Read the model definition and answer for the solid it produces. Units are mm, in the model's axes. A direction names the side the tool comes from. Give positions to 0.01 mm unless a question says otherwise; leave off trailing zeros. Write each loop counter-clockwise with the first axis right and the second up, starting at its lowest first coordinate (ties: lowest second). Pieces come first, ordered by that corner, then holes. Notation, with made-up numbers: M 9,12 L 47,12 A6 ccw 47,20 Z; hole C 75,-2.75 d8. An arc over 180 degrees is marked long. Use a Markdown table: item, result. Add a question column.
Item 1: A cutting plane is placed at C-C on x = 159. Determine the outline of the cut face in (y, z), then the cut area to 3 significant figures.
Item 2: The mould has two halves that part along X. Classify faces 6 (the flat face through (85, 104, 25)), 7 (the cylindrical face through (111.23, 152.4, 19.15)), 8 (the cylindrical face through (20, 13, 75)), 9 (the conical face through (78.414, 33.759, 98.87)): pulls with the +X half, pulls with the -X half, needs draft (parallel to the pull), parting line crosses it, or undercut.
Item 3: For faces 1 (the flat face through (35, 15, 74)), 2 (the flat face through (203, 13, 80)), 3 (the flat face through (25, 37, 74)), 4 (the cylindrical face through (32.69, 42.4, 68.46)), 5 (the flat face through (185, 38, 74)), determine the directions among +Z, -Z, +X, -X, +Y, -Y from which every point of the face is accessible in a straight line to the end or side of a thin tool.
Item 4: Consider probe 1 along Z at (x, y) = (35, 47); probe 2 along Z at (x, y) = (177, 46); probe 3 along X at (y, z) = (43, 99). Determine where each line is inside the solid, lowest interval first. Write a range as [from, to].
Item 5: Given P1, Ø10, axis at x = 121, z = 33, coming from the +Y side; P2, Ø4.5, axis at x = 94, z = 69, coming from the +Y side; P3, Ø8, axis at x = 78, z = 99, coming from the -Y side; P4, Ø7.5, axis at x = 6, y = 15.5, coming from the -Z side, each flat-ended and moving along its own axis, determine where each tip first touches the part or whether it passes through.
Item 6: A cutting plane is placed at A-A on z = 40. Determine the outline of the cut face in (x, y).
Item 7: A cutting plane is placed at B-B on z = 120. Determine the outline of the cut face in (x, y), then the cut area to 3 significant figures.
from build123d import *

# Parameters (mm, degrees)
BOSS_EXTRUDE1_DEPTH        = 150
CUT_EXTRUDE1_DEPTH         = 260.277843249
M6_TAPPED_HOLE1_D          = 5
M6_TAPPED_HOLE1_DEPTH      = 15
M6_TAPPED_HOLE1_TIP        = 1.502151548
SKETCH13_W                 = 80
SKETCH13_H                 = 25
BOSS_EXTRUDE2_DEPTH        = 110
M6_TAPPED_HOLE2_D          = 5
M6_TAPPED_HOLE2_DEPTH      = 15
M6_TAPPED_HOLE2_TIP        = 1.502151548
F_6_0MM_DOWEL_HOLE_1_D     = 6
F_6_0MM_DOWEL_HOLE_1_DEPTH = 15
F_6_0MM_DOWEL_HOLE_1_TIP   = 1.802581857
SKETCH20_W                 = 6.227014718
SKETCH20_H                 = 4.395715082
BOSS_EXTRUDE3_DEPTH        = 25


with BuildPart() as part:
    # Sketch1 → Boss-Extrude1 (new body)
    with BuildSketch(Plane.XY):
        Polygon((0, 0), (0, 25), (25, 25), (25, 50), (185, 50), (185, 25), (210, 25), (210, 0), (175, 0), (175, 30), (35, 30), (35, 0), align=None)
    extrude(amount=BOSS_EXTRUDE1_DEPTH)

    # Sketch9 → Cut-Extrude1 (cut, through all)
    with BuildSketch(Plane(origin=(0, 25, 0), x_dir=(1, 0, 0), z_dir=(0, 1, 0))):
        with BuildLine():
            Line((210, -70), (210, -80))
            Line((210, -80), (195, -80))
            ThreePointArc((195, -80), (190, -75), (195, -70))
            Line((195, -70), (210, -70))
        make_face()
        with BuildLine():
            Line((15, -70), (0, -70))
            Line((0, -70), (0, -80))
            Line((0, -80), (15, -80))
            ThreePointArc((15, -80), (20, -75), (15, -70))
        make_face()
    extrude(amount=-CUT_EXTRUDE1_DEPTH, mode=Mode.SUBTRACT)

    # M6 Tapped Hole1
    with Locations(Plane(origin=(0, 50, 0), x_dir=(1, 0, 0), z_dir=(0, 1, 0))):
        with Locations((35, -82.5), (35, -67.5), (50, -67.5), (50, -82.5), (78, -69), (78, -99), (94, -69), (94, -99), (177.5, -97), (177.5, -53)):
            Hole(M6_TAPPED_HOLE1_D / 2, depth=M6_TAPPED_HOLE1_DEPTH)
            with Locations((0, 0, -(M6_TAPPED_HOLE1_DEPTH + M6_TAPPED_HOLE1_TIP / 2))):  # 118° drill point
                Cone(0, M6_TAPPED_HOLE1_D / 2, M6_TAPPED_HOLE1_TIP, mode=Mode.SUBTRACT)

    # Sketch13 → Boss-Extrude2 (add)
    with BuildSketch(Plane(origin=(0, 50, 0), x_dir=(1, 0, 0), z_dir=(0, 1, 0))):
        with Locations((86, -12.5)):
            Rectangle(SKETCH13_W, SKETCH13_H)
    extrude(amount=BOSS_EXTRUDE2_DEPTH)

    # M6 Tapped Hole2
    with Locations(Plane(origin=(0, 160, 0), x_dir=(1, 0, 0), z_dir=(0, 1, 0))):
        with Locations((58, -18), (114, -8)):
            Hole(M6_TAPPED_HOLE2_D / 2, depth=M6_TAPPED_HOLE2_DEPTH)
            with Locations((0, 0, -(M6_TAPPED_HOLE2_DEPTH + M6_TAPPED_HOLE2_TIP / 2))):  # 118° drill point
                Cone(0, M6_TAPPED_HOLE2_D / 2, M6_TAPPED_HOLE2_TIP, mode=Mode.SUBTRACT)

    # Ø6.0mm dowel hole 1
    with Locations(Plane(origin=(0, 160, 0), x_dir=(1, 0, 0), z_dir=(0, 1, 0))):
        with Locations((58, -8), (114, -18)):
            Hole(F_6_0MM_DOWEL_HOLE_1_D / 2, depth=F_6_0MM_DOWEL_HOLE_1_DEPTH)
            with Locations((0, 0, -(F_6_0MM_DOWEL_HOLE_1_DEPTH + F_6_0MM_DOWEL_HOLE_1_TIP / 2))):  # 118° drill point
                Cone(0, F_6_0MM_DOWEL_HOLE_1_D / 2, F_6_0MM_DOWEL_HOLE_1_TIP, mode=Mode.SUBTRACT)

    # Sketch20 → Boss-Extrude3 (add)
    with BuildSketch(Plane.XY.offset(25)):
        with Locations((85.142135624, 59.920221849)):
            Rectangle(SKETCH20_W, SKETCH20_H)
    extrude(amount=BOSS_EXTRUDE3_DEPTH)


solid = part.part
Filled in:
| question | item | result |
|---|---|---|
| 1 | outline | M 30,0 L 50,0 L 50,150 L 30,150 Z |
| 1 | area | 3,000 mm² |
| 2 | face 6 | needs draft |
| 2 | face 7 | undercut |
| 2 | face 8 | pulls with the -X half |
| 2 | face 9 | undercut |
| 3 | face 1 | +Z, -Z, -Y |
| 3 | face 2 | +X, +Y, -Y |
| 3 | face 3 | +Z, -Z, -X, +Y |
| 3 | face 4 | +Y |
| 3 | face 5 | +Z, -Z, +X, +Y |
| 4 | probe 1 | [0, 65], [70, 80], [85, 150] |
| 4 | probe 2 | [0, 50.55], [55.45, 94.55], [99.45, 150] |
| 4 | probe 3 | [25, 75.5], [80.5, 91.5], [96.5, 176], [179, 185] |
| 5 | P1 | y = 50 |
| 5 | P2 | y = 34.85 |
| 5 | P3 | y = 30 |
| 5 | P4 | z = 0 |
| 6 | outline | M 0,0 L 35,0 L 35,30 L 175,30 L 175,0 L 210,0 L 210,25 L 185,25 L 185,50 L 25,50 L 25,25 L 0,25 Z; M 82.03,57.72 L 88.26,57.72 L 88.26,62.12 L 82.03,62.12 Z |
| 7 | outline | M 0,0 L 35,0 L 35,30 L 175,30 L 175,0 L 210,0 L 210,25 L 185,25 L 185,50 L 25,50 L 25,25 L 0,25 Z |
| 7 | area | 5,050 mm² |
